For this review, take the finished solid that the model builds, in its own axes (mm). Face numbers are marked on the shaded views. Coordinates: 2 decimals unless noted, no trailing zeros. Order: outer loops, then holes, each group sorted by start corner. A loop starts at its lowest first (then second) coordinate and runs counter-clockwise, first axis right, second up. Notation, with made-up numbers: (20.25, 62.5) -> (74.25, 62.5) arc R22 cw to (74.25, 91.5) -> close; hole circle Ø5 at (-24, -3). An arc over 180 degrees is marked (long way). Answer as a JSON object with one key per item and string values. Group by question number.
1) Add section A-A, the plane x = 0. Write out the cut boundary in (y, z).
2) Add section B-B, the plane y = 58. Write out the cut boundary in (x, z), then the cut area to 3 significant figures.
3) Draft analysis for pull direction Y (two halves, no side actions). For the marked faces 1, 2 and 3, state which applies: +Y half, -Y half, draft (parallel to the pull), parting line (faces both ways), or undercut.
4) Add section C-C, the plane x = -70. Write out the cut boundary in (y, z), then the cut area to 3 significant figures.
5) Wall thickness on L1, parallel to Y at x = -70, z = 4.2; L2, parallel to X at y = 58, z = 3.05; L3, parallel to X at y = 58, z = 12.5: over which ranges is each line inside the solid? List them lowest first.
6) Add section D-D, the plane y = 0. Write out the cut boundary in (x, z), then the cut area to 3 significant figures.
7) For pin 1 (13.5 mm diameter, centred on x = 70, y = 0, fed in from +Z), flat-tipped, find the tip position at first contact; note if it passes through.
from build123d import *

# Parameters (mm, degrees)
SKETCH1_R                                            = 55.5
BOSS_EXTRUDE1_DEPTH                                  = 15
CIRPATTERN1_COUNT                                    = 4
HOLE_SIZE_PER_SOCKET_HEAD_CAP_SCREW_TYPE_D           = 9
HOLE_SIZE_PER_SOCKET_HEAD_CAP_SCREW_TYPE_CBORE_D     = 15
HOLE_SIZE_PER_SOCKET_HEAD_CAP_SCREW_TYPE_CBORE_DEPTH = 9


with BuildPart() as part:
    # Sketch1 → Boss-Extrude1 (new body)
    with BuildSketch(Plane.XY):
        Polygon((-80, 65), (-75, 70), (75, 70), (80, 65), (80, -65), (75, -70), (-75, -70), (-80, -65), align=None)
        Circle(SKETCH1_R, mode=Mode.SUBTRACT)
    extrude(amount=BOSS_EXTRUDE1_DEPTH)

    # Sketch2 → M8 Tapped Hole1 (revolve, cut)
    with BuildSketch(Plane(origin=(51.265241636, 51.265241636, 15), x_dir=(0, -1, 0), z_dir=(1, 0, 0))):
        Polygon((0, 0), (0, 21.792926105), (3.4, 19.75), (3.4, 0), align=None)
    m8_tapped_hole1 = revolve(axis=Axis((51.265241636, 51.265241636, 21.35), (0, 0, -1)), mode=Mode.SUBTRACT)

    # CirPattern1: M8 Tapped Hole1 ×4 about axis
    cirpattern1_axis = Axis((0, 0, 0), (0, 0, 1))
    for i in range(1, CIRPATTERN1_COUNT):
        add(m8_tapped_hole1.rotate(cirpattern1_axis, i * 360 / CIRPATTERN1_COUNT), mode=Mode.SUBTRACT)

    # Hole size per socket head cap screw type1 (through all)
    with Locations(Plane(origin=(37.833357844, 52.116019714, 15), x_dir=(-1, 0, 0), z_dir=(0, 0, 1))):
        with Locations((-32.166642156, -5.883980286), (-32.166642156, 52.116019714), (-32.166642156, 110.116019714)):
            hole_size_per_socket_head_cap_screw_type = CounterBoreHole(HOLE_SIZE_PER_SOCKET_HEAD_CAP_SCREW_TYPE_D / 2, HOLE_SIZE_PER_SOCKET_HEAD_CAP_SCREW_TYPE_CBORE_D / 2, HOLE_SIZE_PER_SOCKET_HEAD_CAP_SCREW_TYPE_CBORE_DEPTH)

    # Mirror1: Hole size per socket head cap screw type1 across plane
    add(hole_size_per_socket_head_cap_screw_type.mirror(Plane(origin=(0, 0, 0), x_dir=(0, 0, 1), z_dir=(1, 0, 0))), mode=Mode.SUBTRACT)


solid = part.part
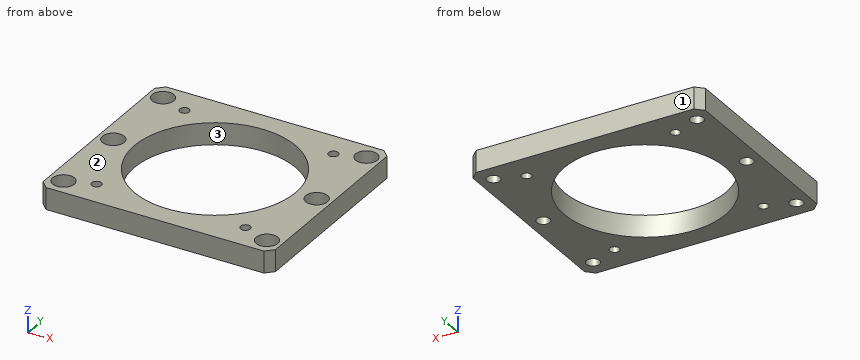
Output values:
{
 "1": {"outline": "(-70, 0) -> (-55.5, 0) -> (-55.5, 15) -> (-70, 15) -> close; (55.5, 0) -> (70, 0) -> (70, 15) -> (55.5, 15) -> close"},
 "2": {"outline": "(-80, 0) -> (-74.5, 0) -> (-74.5, 6) -> (-77.5, 6) -> (-77.5, 15) -> (-80, 15) -> close; (-65.5, 0) -> (65.5, 0) -> (65.5, 6) -> (62.5, 6) -> (62.5, 15) -> (-62.5, 15) -> (-62.5, 6) -> (-65.5, 6) -> close; (74.5, 0) -> (80, 0) -> (80, 15) -> (77.5, 15) -> (77.5, 6) -> (74.5, 6) -> close", "area": "2,020 mm²"},
 "3": {"face 1": "+Y half", "face 2": "draft", "face 3": "undercut"},
 "4": {"outline": "(-70, 0) -> (-62.5, 0) -> (-62.5, 6) -> (-65.5, 6) -> (-65.5, 15) -> (-70, 15) -> close; (-53.5, 0) -> (-4.5, 0) -> (-4.5, 6) -> (-7.5, 6) -> (-7.5, 15) -> (-50.5, 15) -> (-50.5, 6) -> (-53.5, 6) -> close; (4.5, 0) -> (53.5, 0) -> (53.5, 6) -> (50.5, 6) -> (50.5, 15) -> (7.5, 15) -> (7.5, 6) -> (4.5, 6) -> close; (62.5, 0) -> (70, 0) -> (70, 15) -> (65.5, 15) -> (65.5, 6) -> (62.5, 6) -> close", "area": "1,530 mm²"},
 "5": {"L1": "y = -70 to -62.5, -53.5 to -4.5, 4.5 to 53.5, 62.5 to 70", "L2": "x = -80 to -74.5, -65.5 to 65.5, 74.5 to 80", "L3": "x = -80 to -77.5, -62.5 to 62.5, 77.5 to 80"},
 "6": {"outline": "(-80, 0) -> (-74.5, 0) -> (-74.5, 6) -> (-77.5, 6) -> (-77.5, 15) -> (-80, 15) -> close; (-65.5, 0) -> (-55.5, 0) -> (-55.5, 15) -> (-62.5, 15) -> (-62.5, 6) -> (-65.5, 6) -> close; (55.5, 0) -> (65.5, 0) -> (65.5, 6) -> (62.5, 6) -> (62.5, 15) -> (55.5, 15) -> close; (74.5, 0) -> (80, 0) -> (80, 15) -> (77.5, 15) -> (77.5, 6) -> (74.5, 6) -> close", "area": "357 mm²"},
 "7": {"pin 1": "stops at z = 6"}
}
